The listing builds one solid part. Answer for the finished solid, in the listing's coordinates (mm). A direction names the side the tool comes from. Coordinates: 2 decimals unless noted, no trailing zeros. Loops run counter-clockwise (first coordinate to the right, second up) from the corner with the lowest first, then second, coordinate; pieces in that order, holes last. Notation, with made-up numbers: (47.5, 66.5) - (83.5, 66.5) arc R26 cw to (83.5, 80.5) - close; hole circle Ø1 at (40, 3.25). An arc over 180 degrees is marked (long way). Return JSON: item names as keys, results as strings. Group by question number.
1. Section A-A (z = 280.5) is taken. Write down the section's boundary in (x, y).
2. Each of these flat-tipped pins is pushed along its axis until it touches: P1, Ø1, axis at x = -1.5, y = -2.5, coming from the +Z side; P2, Ø4, axis at y = 5.5, z = 332, coming from the -X side; P3, Ø4, axis at y = 6.5, z = 132, coming from the -X side. Where does it stop, or does it pass through?
3. Which of the six approach directions +Z, -Z, +X, -X, +Y, -Y give full straight-line access (tool end or side, diameter ignored) to faces 5 (the face through (-0.704, 0.222, 34.11)), 6 (the face through (-2.285, 3.584, 507.578))?
4. Find the intervals of material crossed by line 1 along Y through (x, z) = (0, 10); line 2 along Y through (x, z) = (2, 47); line 3 along X through (y, z) = (-1.5, 25.5), in increasing order.
5. The mould has two halves that part along Y. Classify faces 1 (the face through (-0.16, -0.72, 493.39)), 2 (the face through (-4.336, -19.524, 256.374)), 3 (the face through (-0.3, 4.5, 520)), 4 (the face through (2.285, 3.584, 16.224)): pulls with the +Y half, pulls with the -Y half, needs draft (parallel to the pull), parting line crosses it, or undercut.
```python
from build123d import *

# Parameters (mm, degrees)
SKETCH_1_R              = 20
EXTRUDE_1_DEPTH         = 520
HOLE_WIZARD_M10_1_D     = 8.5
HOLE_WIZARD_M10_1_DEPTH = 32
HOLE_WIZARD_M10_1_TIP   = 2.553657631
CHAMFER_1_SIZE          = 1
CHAMFER_2_SIZE          = 1
HOLE_WIZARD_M10_2_D     = 8.5
HOLE_WIZARD_M10_2_DEPTH = 24.5
HOLE_WIZARD_M10_2_TIP   = 2.553657631


with BuildPart() as part:
    # 草图1 → 凸台-拉伸1 (new body)
    with BuildSketch(Plane.XY):
        Circle(SKETCH_1_R)
    extrude(amount=EXTRUDE_1_DEPTH)

    # M10 螺纹孔1
    with Locations(Plane(origin=(0, 0, 0), x_dir=(-1, 0, 0), z_dir=(0, 0, -1))):
        with Locations((0, 0)):
            Hole(HOLE_WIZARD_M10_1_D / 2, depth=HOLE_WIZARD_M10_1_DEPTH)
            with Locations((0, 0, -(HOLE_WIZARD_M10_1_DEPTH + HOLE_WIZARD_M10_1_TIP / 2))):  # 118° drill point
                Cone(0, HOLE_WIZARD_M10_1_D / 2, HOLE_WIZARD_M10_1_TIP, mode=Mode.SUBTRACT)

    # 倒角1
    chamfer_1_edges = [part.edges().sort_by_distance(p)[0] for p in [
        (-20, 0, 520),
    ]]
    chamfer(chamfer_1_edges, length=CHAMFER_1_SIZE)

    # 倒角2
    chamfer_2_edges = [part.edges().sort_by_distance(p)[0] for p in [
        (-20, 0, 0),
    ]]
    chamfer(chamfer_2_edges, length=CHAMFER_2_SIZE)

    # M10 螺纹孔2
    with Locations(Plane.XY.offset(520)):
        with Locations((0, 0)):
            Hole(HOLE_WIZARD_M10_2_D / 2, depth=HOLE_WIZARD_M10_2_DEPTH)
            with Locations((0, 0, -(HOLE_WIZARD_M10_2_DEPTH + HOLE_WIZARD_M10_2_TIP / 2))):  # 118° drill point
                Cone(0, HOLE_WIZARD_M10_2_D / 2, HOLE_WIZARD_M10_2_TIP, mode=Mode.SUBTRACT)


solid = part.part
```
The answers:
{
 "1": {"outline": "circle Ø40 at (0, 0)"},
 "2": {"P1": "stops at z = 495", "P2": "stops at x = -19.69", "P3": "stops at x = -19.49"},
 "3": {"face 5": "-Z", "face 6": "+Z"},
 "4": {"line 1": "y = -20 to -4.25, 4.25 to 20", "line 2": "y = -19.9 to 19.9", "line 3": "x = -19.94 to -3.98, 3.98 to 19.94"},
 "5": {"face 1": "undercut", "face 2": "parting line crosses it", "face 3": "needs draft", "face 4": "undercut"}
}
